For this review, take the finished solid that the model builds, in its own axes (mm). A direction names the side the tool comes from. Give positions to 0.01 mm unless a question says otherwise; leave off trailing zeros. Write each loop counter-clockwise with the first axis right and the second up, starting at its lowest first coordinate (ties: lowest second). Pieces come first, ordered by that corner, then holes. Notation, with made-up numbers: M 63,54 L 116,54 A36 ccw 116,90 Z; hole C 63.25,38 d4. An arc over 180 degrees is marked long. Write item = value, one per line.
```python
from build123d import *

# Parameters (mm, degrees)
SKETCH_1_W                = 15
SKETCH_1_H                = 10
EXTRUDE_1_DEPTH           = 6.5
HOLE_WIZARD_1_D           = 4.5
HOLE_WIZARD_1_CBORE_D     = 8
HOLE_WIZARD_1_CBORE_DEPTH = 4.6


with BuildPart() as part:
    # 草图1 → 凸台-拉伸1 (new, symmetric)
    with BuildSketch(Plane(origin=(0, 0, 0), x_dir=(1, 0, 0), z_dir=(0, 1, 0))):
        Rectangle(SKETCH_1_W, SKETCH_1_H)
    extrude(amount=EXTRUDE_1_DEPTH, both=True)

    # 打孔尺寸(%根据)内六角圆柱头螺钉的类型1 (through all)
    with Locations(Plane(origin=(0, 6.5, 0), x_dir=(1, 0, 0), z_dir=(0, 1, 0))):
        with Locations((0, 0)):
            CounterBoreHole(HOLE_WIZARD_1_D / 2, HOLE_WIZARD_1_CBORE_D / 2, HOLE_WIZARD_1_CBORE_DEPTH)


solid = part.part
```
1. Insertion check: P1, Ø5, axis at x = 1.5, z = 3.5, coming from the +Y side; P2, Ø5, axis at x = -1, z = 0, coming from the +Y side; P3, Ø2, axis at x = -0.5, z = 1, coming from the +Y side. Each pin has a flat end and moves straight along its axis. Give the tip position at first contact, or say it passes through.
Responses:
P1 = 6.5
P2 = 1.9
P3 = through
2. We need section C-C, the plane y = 3.25. Write out the cut boundary in (x, z), then the cut area to 3 significant figures.
Responses:
outline = M -7.5,-5 L 7.5,-5 L 7.5,5 L -7.5,5 Z; hole C 0,0 d8
area = 99.7 mm2
3. We need section A-A, the plane z = 0. Write out the cut boundary in (x, y), then the cut area to 3 significant figures.
Responses:
outline = M -7.5,-6.5 L -2.25,-6.5 L -2.25,1.9 L -4,1.9 L -4,6.5 L -7.5,6.5 Z; M 2.25,-6.5 L 7.5,-6.5 L 7.5,6.5 L 4,6.5 L 4,1.9 L 2.25,1.9 Z
area = 120 mm2
4. Machinability: for faces 1 (the face through (7.5, 0, 0)), 2 (the face through (-0.867, 4.232, 3.905)), which of the approach directions +Z, -Z, +X, -X, +Y, -Y give a long, thin tool a straight path to every point of the face, cutting with its end or side? Answer none if there is none.
Responses:
face_1 = +Z, -Z, +X, +Y, -Y
face_2 = +Y
5. The part is to be moulded in two halves that separate along X. For faces 3 (the face through (-7.5, 0, 0)), 4 (the face through (0.29, -2.36, -2.23)), 5 (the face through (-0.1, 6.5, 4.4)), say which applies: +X half, -X half, draft (parallel to the pull), parting line (faces both ways), or undercut.
Responses:
face_3 = -X half
face_4 = undercut
face_5 = draft
6. For line 1 along Z through (x, y) = (0, 5.6); line 2 along Z through (x, y) = (0, -1.5); line 3 along Y through (x, z) = (3.5, 0.75), list the stretches that pass through material, from the lowest coordinate up. Write a range as from..to.
Responses:
line_1 = -5..-4, 4..5
line_2 = -5..-2.25, 2.25..5
line_3 = -6.5..1.9
7. We need section B-B, the plane x = 0. Write out the cut boundary in (y, z), then the cut area to 3 significant figures.
Responses:
outline = M -6.5,-5 L 6.5,-5 L 6.5,-4 L 1.9,-4 L 1.9,-2.25 L -6.5,-2.25 Z; M -6.5,2.25 L 1.9,2.25 L 1.9,4 L 6.5,4 L 6.5,5 L -6.5,5 Z
area = 55.4 mm2
8. We need section D-D, the plane y = -5.25. Write out the cut boundary in (x, z), then the cut area to 3 significant figures.
Responses:
outline = M -7.5,-5 L 7.5,-5 L 7.5,5 L -7.5,5 Z; hole C 0,0 d4.5
area = 134 mm2
